For this review, use the dimensioned drawing (mm, ordinates from the lowest corner) and the shaded views. A direction names the side the tool comes from. Coordinates: 2 decimals unless noted, no trailing zeros. Order: outer loops, then holes, each group sorted by start corner. A loop starts at its lowest first (then second) coordinate and runs counter-clockwise, first axis right, second up. Notation, with made-up numbers: M 44.25,25.5 L 61.25,25.5 A33 cw 61.25,55.5 Z; hole C 42.25,-21 d10. An arc over 180 degrees is marked long. Answer in a Markdown table with one row per item.
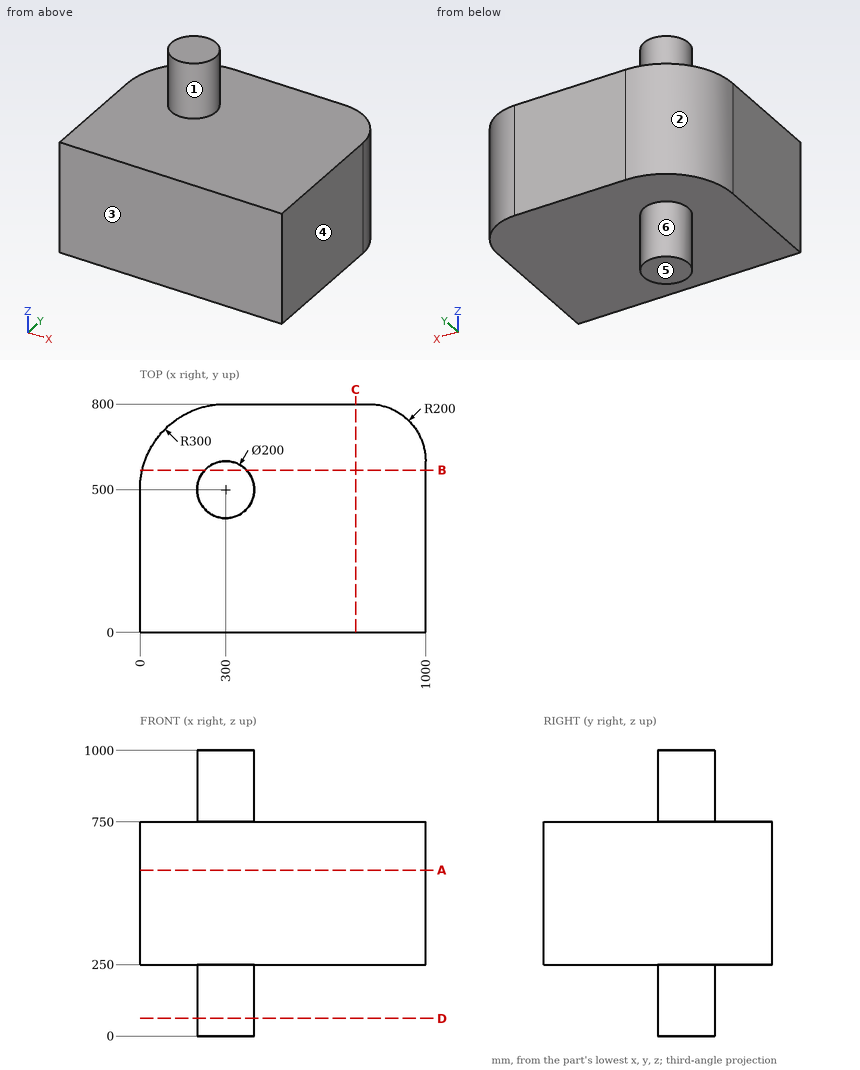
(1) Insertion check: pin 1 Ø4 at (x, y) = (849, 216) entering from -Z; pin 2 Ø3 at (y, z) = (634, 623) entering from +X; pin 3 Ø1 at (x, y) = (505.5, 553.5) entering from +Z. Each pin has a flat end and moves straight along its axis. Give the tip position at first contact, or say it passes through.
Return value:
| item | result |
|---|---|
| pin 1 | stops at z = 250 |
| pin 2 | stops at x = 997.34 |
| pin 3 | stops at z = 750 |
(2) For line 1 along Z through (x, y) = (382.5, 399); line 2 along Y through (x, z) = (298.5, 126.5); line 3 along X through (y, z) = (654, 352), list the stretches that pass through material, from the lowest coordinate up. Write a range as from..to.
Return value:
| item | result |
|---|---|
| line 1 | z = 250..750 |
| line 2 | y = 400.01..599.99 |
| line 3 | x = 42.54..992.57 |
(3) Draft analysis for pull direction Y (two halves, no side actions). For the marked faces 1, 2, 3 and 4, state which applies: pulls with the +Y half, pulls with the -Y half, needs draft (parallel to the pull), parting line crosses it, or undercut.
Return value:
| item | result |
|---|---|
| face 1 | parting line crosses it |
| face 2 | pulls with the +Y half |
| face 3 | pulls with the -Y half |
| face 4 | needs draft |
(4) For the marked faces 5 and 6, list the 3-axis set-ups (+Z, -Z, +X, -X, +Y, -Y) from which the entire face can be reached by the end or side of a thin tool; tool diameter is ignored.
Return value:
| item | result |
|---|---|
| face 5 | -Z, +X, -X, +Y, -Y |
| face 6 | -Z |
(5) Add section D-D, the plane z = 61.5. Give the boundary of the cut face in (x, y), and give its area (3 significant figures).
Return value:
| item | result |
|---|---|
| outline | C 300,500 d200 |
| area | 31,400 mm2 |
(6) Add section A-A, the plane z = 581. Give the boundary of the cut face in (x, y).
Return value:
| item | result |
|---|---|
| outline | M 0,0 L 1000,0 L 1000,600 A200 ccw 800,800 L 300,800 A300 ccw 0,500 Z |
(7) Add section B-B, the plane y = 568.5. Give the boundary of the cut face in (x, z), and give its area (3 significant figures).
Return value:
| item | result |
|---|---|
| outline | M 7.93,250 L 227.15,250 L 227.15,0 L 372.85,0 L 372.85,250 L 1000,250 L 1000,750 L 372.85,750 L 372.85,1000 L 227.15,1000 L 227.15,750 L 7.93,750 Z |
| area | 569,000 mm2 |
(8) Add section C-C, the plane x = 755. Give the boundary of the cut face in (y, z).
Return value:
| item | result |
|---|---|
| outline | M 0,250 L 800,250 L 800,750 L 0,750 Z |
